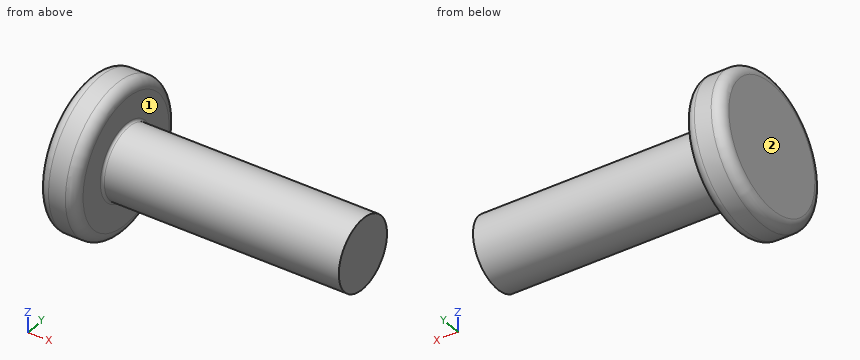
```python
from build123d import *


with BuildPart() as part:
    # Dimensioned Sketch → Revolve3 (revolve)
    with BuildSketch(Plane.XY, mode=Mode.PRIVATE) as revolve3_sk:
        with BuildLine():
            Line((0, 0), (0, 2.6752))
            ThreePointArc((0, 2.6752), (0.130278904, 2.989721096), (0.4448, 3.12))
            Line((0.4448, 3.12), (1.1552, 3.12))
            ThreePointArc((1.1552, 3.12), (1.469721096, 2.989721096), (1.6, 2.6752))
            Line((1.6, 2.6752), (1.6, 1.6))
            ThreePointArc((1.6, 1.6), (1.629289322, 1.529289322), (1.7, 1.5))
            Line((1.7, 1.5), (11.6, 1.5))
            Line((11.6, 1.5), (11.6, 0))
            Line((11.6, 0), (0, 0))
        make_face()
    revolve(revolve3_sk.sketch.rotate(Axis((0, 0, 0), (1, 0, 0)), 90), axis=Axis((0, 0, 0), (1, 0, 0)))


solid = part.part
```
The listing builds one solid part. Answer for the finished solid, in the listing's coordinates (mm). Face numbers are marked on the shaded views. A direction names the side the tool comes from. Give positions to 0.01 mm unless a question says otherwise; leave off trailing zeros. Order: outer loops, then holes, each group sorted by start corner. A loop starts at its lowest first (then second) coordinate and runs counter-clockwise, first axis right, second up. Notation, with made-up numbers: (70, 80) - (108, 80) arc R20 ccw to (108, 111) - close; hole circle Ø10 at (58, 59.5). An arc over 180 degrees is marked (long way). Answer in a Markdown table with one row per item. Add a question column.
Q1. Given P1, Ø3, axis at x = 2.5, z = -2, coming from the +Y side; P2, Ø3, axis at y = -1.5, z = 1.5, coming from the +X side; P3, Ø3, axis at x = 6, z = -2.5, coming from the -Y side, each flat-ended and moving along its own axis, determine where each tip first touches the part or whether it passes through.
Q2. The part is cut by section A-A (y = 0). Determine the outline of the cut face in (x, z).
Q3. Which of the six approach directions +Z, -Z, +X, -X, +Y, -Y give full straight-line access (tool end or side, diameter ignored) to the marked faces 1 and 2?
Q4. Find the intervals of material crossed by line 1 along X through (y, z) = (-2, -0.75); line 2 along Y through (x, z) = (2.75, 0); line 3 along X through (y, z) = (1.75, 2.5), in increasing order. Write a range as [from, to].
Q5. The part is cut by section C-C (x = 8). Determine the outline of the cut face in (y, z), then the cut area to 3 significant figures.
Determined:
| question | item | result |
|---|---|---|
| 1 | P1 | stops at y = 2.9 |
| 1 | P2 | stops at x = 11.6 |
| 1 | P3 | stops at y = -1.12 |
| 2 | outline | (0, -2.68) arc R0.44 ccw to (0.44, -3.12) - (1.16, -3.12) arc R0.44 ccw to (1.6, -2.68) - (1.6, -1.6) arc R0.1 cw to (1.7, -1.5) - (11.6, -1.5) - (11.6, 1.5) - (1.7, 1.5) arc R0.1 cw to (1.6, 1.6) - (1.6, 2.68) arc R0.44 ccw to (1.16, 3.12) - (0.44, 3.12) arc R0.44 ccw to (0, 2.68) - close |
| 3 | face 1 | +X |
| 3 | face 2 | +Z, -Z, -X, +Y, -Y |
| 4 | line 1 | x = [0, 1.6] |
| 4 | line 2 | y = [-1.5, 1.5] |
| 4 | line 3 | x = [0.21, 1.39] |
| 5 | outline | circle Ø3 at (0, 0) |
| 5 | area | 7.07 mm² |
